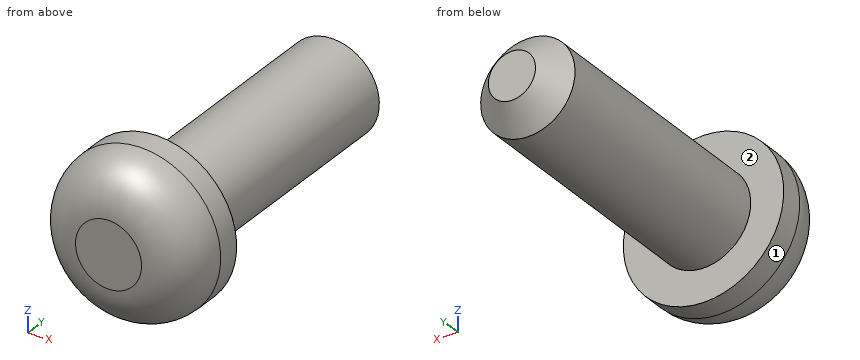
```python
from build123d import *

# Parameters (mm, degrees)
SKETCH1_R           = 1
BOSS_EXTRUDE1_DEPTH = 6
CHAMFER1_SIZE       = 0.5
SKETCH2_R           = 1.7
BOSS_EXTRUDE2_DEPTH = 1.5
FILLET1_R           = 1


with BuildPart() as part:
    # Sketch1 → Boss-Extrude1 (new body)
    with BuildSketch(Plane(origin=(0, 0, 0), x_dir=(1, 0, 0), z_dir=(0, 1, 0))):
        with Locations(Location((0, 0, 0), (0, 0, 270))):
            Circle(SKETCH1_R)
    extrude(amount=BOSS_EXTRUDE1_DEPTH)

    # Chamfer1
    chamfer1_edges = [part.edges().sort_by_distance(p)[0] for p in [
        (0, 6, -1),
    ]]
    chamfer(chamfer1_edges, length=CHAMFER1_SIZE)

    # Sketch2 → Boss-Extrude2 (add)
    with BuildSketch(Plane.XZ):
        with Locations(Location((0, 0, 0), (0, 0, 270))):
            Circle(SKETCH2_R)
    extrude(amount=BOSS_EXTRUDE2_DEPTH)

    # Fillet1
    fillet1_edges = [part.edges().sort_by_distance(p)[0] for p in [
        (0, -1.5, 1.7),
    ]]
    fillet(fillet1_edges, radius=FILLET1_R)


solid = part.part
```
CAD build for the part. Positions are in the model's coordinates, mm. Face numbers are marked on the shaded views. A direction names the side the tool comes from. Coordinates: 2 decimals unless noted, no trailing zeros. Order: outer loops, then holes, each group sorted by start corner. A loop starts at its lowest first (then second) coordinate and runs counter-clockwise, first axis right, second up. Notation, with made-up numbers: (87.5, 15.25) -> (143.5, 15.25) arc R18 ccw to (143.5, 26.25) -> close; hole circle Ø4 at (-16, 42.25). An arc over 180 degrees is marked (long way). Use one line per item in the form item = value. Start each with the question number.
1) Drill centre lines: L1, parallel to Z at x = 0.25, y = 2; L2, parallel to Y at x = 0.35, z = 0.4; L3, parallel to Y at x = -0.9, z = 0.85. Where is each one in solid material? Low to high. Write a range as [from, to].
2) Band-saw the part on A-A on y = 0.5. Give the cut face in (x, z).
3) Tool access for the marked faces 1 and 2: list every direction of +Z, -Z, +X, -X, +Y, -Y with a clear straight run to the whole face (end or side of a thin tool).
4) Drop flat-ended pins along their axis: pin 1 (1 mm diameter, centred on x = 0.5, y = 3.5, fed in from +Z); pin 2 (1 mm diameter, centred on y = -0.5, z = 1, fed in from +X). Give the stop position or say it passes through.
Entries:
q1.L1 = [-0.97, 0.97]
q1.L2 = [-1.5, 5.97]
q1.L3 = [-1.34, 0]
q2.outline = circle Ø2 at (0, 0)
q3.face_1 = +Y, -Y
q3.face_2 = +Y
q4.pin_1 = 1
q4.pin_2 = 1.62
